Verification items for the finished model (mm, model axes). Face numbers are marked on the shaded views. A direction names the side the tool comes from. Coordinates: 2 decimals unless noted, no trailing zeros. Write each loop counter-clockwise with the first axis right and the second up, starting at its lowest first coordinate (ties: lowest second). Pieces come first, ordered by that corner, then holes. Notation, with made-up numbers: (20.25, -18.75) -> (59.25, -18.75) arc R25 ccw to (59.25, 5.25) -> close; hole circle Ø5 at (82, 10). An arc over 180 degrees is marked (long way). Write each question's results on one line, items separated by ' | '. Start each with the question number.
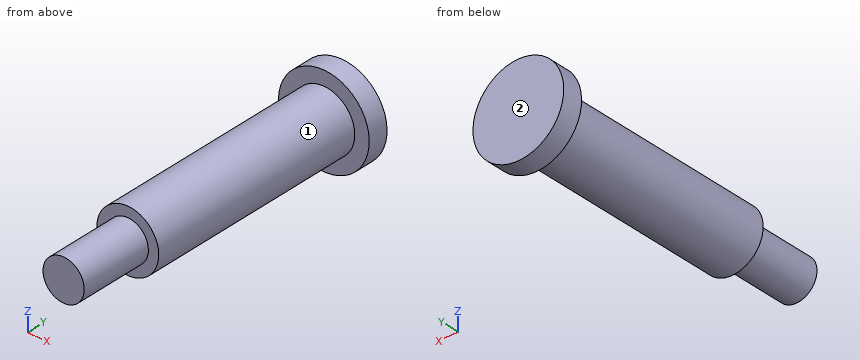
from build123d import *


with BuildPart() as part:
    # Pin Profile Sketch → Pin Body Revolve (revolve)
    with BuildSketch(Plane.XY, mode=Mode.PRIVATE) as pin_body_revolve_sk:
        Polygon((0, 0), (-11, 0), (-11, -5), (-7.5, -5), (-7.5, -60), (-5, -60), (-5, -78), (0, -78), align=None)
    revolve(pin_body_revolve_sk.sketch.rotate(Axis((0, 16.243243243, 0), (0, -1, 0)), 270), axis=Axis((0, 16.243243243, 0), (0, -1, 0)))


solid = part.part
1. Sectioned sample at D-D on y = -15. Record the cut outline in (x, z), plus the area to 3 significant figures.
2. Material ranges on probe 1 along Y at (x, z) = (-8.25, 2.25); probe 2 along X at (y, z) = (-68, -0.5); probe 3 along X at (y, z) = (-51, -3.75), recorded low to high. Write a range as from..to.
3. Sectioned sample at A-A on z = 0. Record the cut outline in (x, y), plus the area to 4 significant figures.
4. Tool access check on the marked faces 1 and 2. Record the directions out of +Z, -Z, +X, -X, +Y, -Y that give a thin tool (end or side, any length) a straight path to the whole face; none if there is none.
5. Sectioned sample at C-C on y = -69. Record the cut outline in (x, z), plus the area to 3 significant figures.
6. Sectioned sample at B-B on x = 0. Record the cut outline in (y, z).
7. Depth check by flat-ended pin: pin 1 Ø1.5 at (x, y) = (-1.5, -66) entering from +Z; pin 2 Ø10 at (y, z) = (-56, 2.5) entering from -X; pin 3 Ø10 at (x, y) = (-5.5, -61) entering from -Z. Enter the tip coordinate at first touch or a pass-through.
Computed values:
1) outline: circle Ø15 at (0, 0) | area: 177 mm^2
2) probe 1: y = -5..0 | probe 2: x = -4.97..4.97 | probe 3: x = -6.5..6.5
3) outline: (-11, -5) -> (-7.5, -5) -> (-7.5, -60) -> (-5, -60) -> (-5, -78) -> (5, -78) -> (5, -60) -> (7.5, -60) -> (7.5, -5) -> (11, -5) -> (11, 0) -> (-11, 0) -> close | area: 1,115 mm^2
4) face 1: -Y | face 2: +Z, -Z, +X, -X, +Y
5) outline: circle Ø10 at (0, 0) | area: 78.5 mm^2
6) outline: (-78, -5) -> (-60, -5) -> (-60, -7.5) -> (-5, -7.5) -> (-5, -11) -> (0, -11) -> (0, 11) -> (-5, 11) -> (-5, 7.5) -> (-60, 7.5) -> (-60, 5) -> (-78, 5) -> close
7) pin 1: stops at z = 4.94 | pin 2: stops at x = -7.5 | pin 3: stops at z = -7.48
